from build123d import *

# Parameters (mm, degrees)
SKETCH_1_W          = 56.8
SKETCH_1_H          = 38
EXTRUDE_1_DEPTH     = 14
CHAMFER_1_SIZE      = 2
SKETCH_2_W          = 2
SKETCH_2_H          = 34
CUT_EXTRUDE_1_DEPTH = 62.508048254


with BuildPart() as part:
    # 草图1 → 凸台-拉伸1 (new, symmetric)
    with BuildSketch(Plane.XY):
        Rectangle(SKETCH_1_W, SKETCH_1_H)
    extrude(amount=EXTRUDE_1_DEPTH, both=True)

    # 倒角1
    chamfer_1_edges = [part.edges().sort_by_distance(p)[0] for p in [
        (28.4, -19, 0),
        (-28.4, -19, 0),
        (-28.4, 19, 0),
        (28.4, 19, 0),
    ]]
    chamfer(chamfer_1_edges, length=CHAMFER_1_SIZE)

    # 草图2 → 切除-拉伸1 (cut, through all)
    with BuildSketch(Plane(origin=(28.4, 0, 0), x_dir=(0, 0, -1), z_dir=(1, 0, 0))):
        with Locations((-13, 0)):
            Rectangle(SKETCH_2_W, SKETCH_2_H)
    extrude(amount=-CUT_EXTRUDE_1_DEPTH, mode=Mode.SUBTRACT)


solid = part.part
Can you work these out from the model? Positions are in its coordinate system, mm. A direction names the side the tool comes from. Coordinates: 2 decimals unless noted, no trailing zeros. Order: outer loops, then holes, each group sorted by start corner. A loop starts at its lowest first (then second) coordinate and runs counter-clockwise, first axis right, second up. Notation, with made-up numbers: (29, -12.75) - (88, -12.75) arc R37 cw to (88, 26.25) - close; hole circle Ø1 at (0.25, 40). An arc over 180 degrees is marked (long way). Answer as a JSON object with one key per item and string values. Group by question number.
Q1. Imagine slicing it at A-A (x = 3.5). Please give me the cut outline in (y, z), and give its area (3 significant figures).
Q2. Will this pin go through, and if not, where does the flat tip stop? P1, Ø1.5, axis at x = -13.5, y = 2, coming from the +Z side.
Q3. Imagine slicing it at B-B (y = 0.5). Please give me the cut outline in (x, z).
Q4. On a 3-axis mill with a long thin cutter (end or side, diameter ignored), from which of +Z, -Z, +X, -X, +Y, -Y can I reach the whole of each face in a straight line? I mean faces 1 (the face through (0, 0, 12)), 2 (the face through (-27.4, 18, 0.2)). Say none if no direction works.
Q5. I need wall thicknesses on line 1 (Z direction, x = 3, y = 0); line 2 (Y direction, x = -11, z = 13.25). Which ranges of each line are inside material? Lowest first, please. Write a range as from..to.
Determined:
{
 "1": {"outline": "(-19, -14) - (19, -14) - (19, 14) - (17, 14) - (17, 12) - (-17, 12) - (-17, 14) - (-19, 14) - close", "area": "996 mm2"},
 "2": {"P1": "stops at z = 12"},
 "3": {"outline": "(-28.4, -14) - (28.4, -14) - (28.4, 12) - (-28.4, 12) - close"},
 "4": {"face 1": "+Z, +X, -X", "face 2": "+Z, -Z, -X, +Y"},
 "5": {"line 1": "z = -14..12", "line 2": "y = -19..-17, 17..19"}
}
